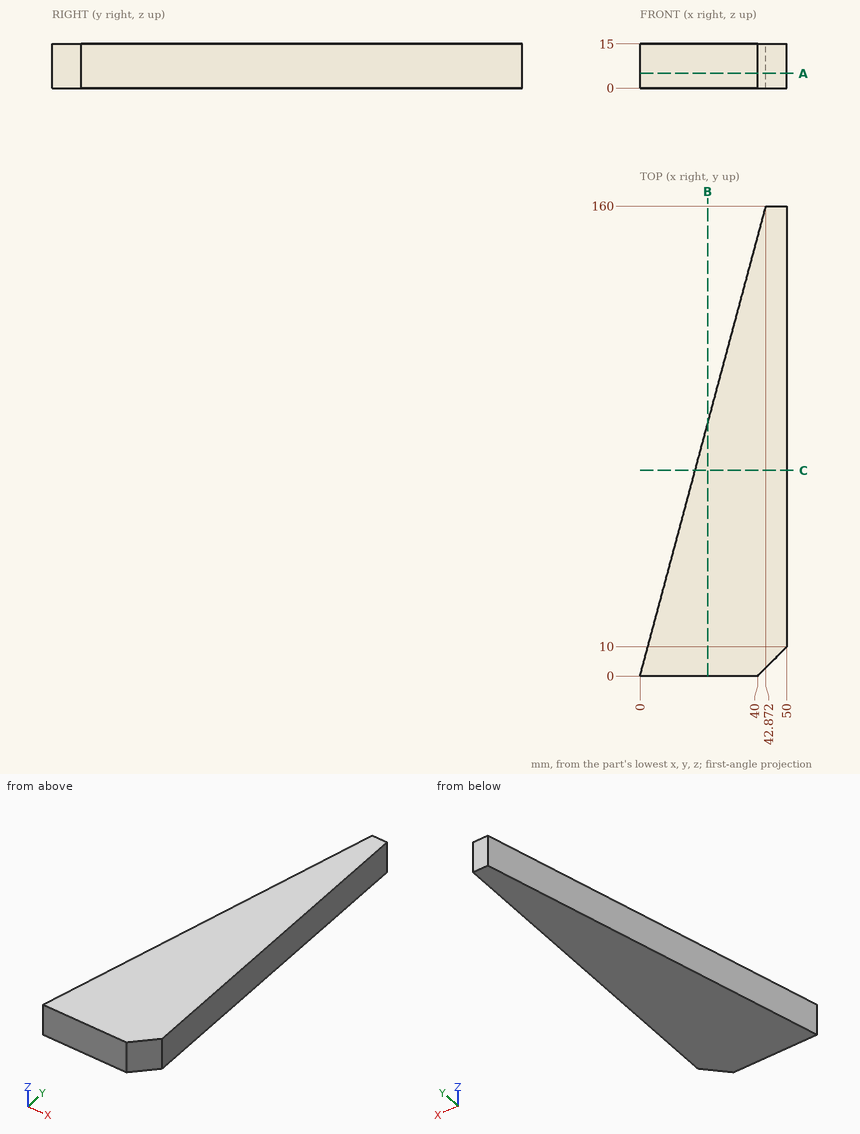
Drawing for the job (mm, zero at the part's lowest x, y, z). Round coordinates to 2 decimals unless told otherwise and drop trailing zeros. Order: outer loops, then holes, each group sorted by start corner. A loop starts at its lowest first (then second) coordinate and runs counter-clockwise, first axis right, second up. Notation, with made-up numbers: M -21.5,51 L -13.5,51 A9 ccw -13.5,61 Z; hole C 15,59.25 d6. An arc over 180 degrees is marked long. Use one line per item in the form item = value.
Q1. Saw through at B-B on x = 23. Give the cut face in (y, z), then the cut area to 3 significant figures.
Recorded:
outline = M 0,0 L 85.84,0 L 85.84,15 L 0,15 Z
area = 1,290 mm^2
Q2. Flat gauge pins, fed straight in: P1, Ø8, axis at y = 61, z = 9, coming from the -X side; P2, Ø1.5, axis at y = 141, z = 7.5, coming from the -X side. Where does each tip first touch, or does it go through?
Recorded:
P1 = 15.27
P2 = 37.58
Q3. Probe L1, parallel to X at y = 59, z = 13.5; L2, parallel to X at y = 41, z = 13.75; L3, parallel to Y at x = 45.5, z = 3. List the from-to ranges inside material, lowest first.
Recorded:
L1 = 15.81 to 50
L2 = 10.99 to 50
L3 = 5.5 to 160
Q4. Saw through at A-A on z = 5. Give the cut face in (x, y).
Recorded:
outline = M 0,0 L 40,0 L 50,10 L 50,160 L 42.87,160 Z
Q5. Saw through at C-C on y = 70. Give the cut face in (x, z), then the cut area to 3 significant figures.
Recorded:
outline = M 18.76,0 L 50,0 L 50,15 L 18.76,15 Z
area = 469 mm^2
